The listing builds one solid part. Answer for the finished solid, in the listing's coordinates (mm). A direction names the side the tool comes from. Give positions to 0.01 mm unless a question says otherwise; leave off trailing zeros. Write each loop counter-clockwise with the first axis right and the second up, starting at its lowest first coordinate (ties: lowest second). Pieces come first, ordered by that corner, then holes.
```python
from build123d import *

# Parameters (mm, degrees)
SKETCH1_W           = 70
SKETCH1_H           = 30
BOSS_EXTRUDE1_DEPTH = 6
SKETCH2_R           = 1.25
CUT_EXTRUDE1_DEPTH  = 5
CUT_EXTRUDE2_START  = -5
SKETCH3_R           = 1.25
CUT_EXTRUDE2_DEPTH  = 5


with BuildPart() as part:
    # Sketch1 → Boss-Extrude1 (new body)
    with BuildSketch(Plane(origin=(0, 0, 0), x_dir=(1, 0, 0), z_dir=(0, 1, 0))):
        Rectangle(SKETCH1_W, SKETCH1_H)
    extrude(amount=BOSS_EXTRUDE1_DEPTH)

    # Sketch2 → Cut-Extrude1 (cut)
    with BuildSketch(Plane(origin=(35, 0, 0), x_dir=(0, 0, -1), z_dir=(1, 0, 0))):
        with Locations((11.5, 3)):
            Circle(SKETCH2_R)
        with Locations((-11.5, 3)):
            Circle(SKETCH2_R)
    extrude(amount=-CUT_EXTRUDE1_DEPTH, mode=Mode.SUBTRACT)

    # Sketch3 → Cut-Extrude2 (cut)
    with BuildSketch(Plane.ZY.offset(35).offset(CUT_EXTRUDE2_START)):
        with Locations(Location((-11.5, 3, 0), (0, 0, 180))):
            Circle(SKETCH3_R)
        with Locations(Location((11.5, 3, 0), (0, 0, 180))):
            Circle(SKETCH3_R)
    extrude(amount=CUT_EXTRUDE2_DEPTH, mode=Mode.SUBTRACT)


solid = part.part
```
Item 1: A cutting plane is placed at A-A, the plane z = 11.5. Give the vertices of the cut face in (x, y), plus the area to 3 significant figures.
Conclusion:
outline: (-35, 0) - (35, 0) - (35, 1.75) - (30, 1.75) - (30, 4.25) - (35, 4.25) - (35, 6) - (-35, 6) - (-35, 4.25) - (-30, 4.25) - (-30, 1.75) - (-35, 1.75) - close
area: 395 mm2
Item 2: A cutting plane is placed at C-C, the plane z = -11.75. Give the vertices of the cut face in (x, y), plus the area to 3 significant figures.
Conclusion:
outline: (-35, 0) - (35, 0) - (35, 1.78) - (30, 1.78) - (30, 4.22) - (35, 4.22) - (35, 6) - (-35, 6) - (-35, 4.22) - (-30, 4.22) - (-30, 1.78) - (-35, 1.78) - close
area: 396 mm2
Item 3: Each of these flat-tipped pins is pushed along its axis until it touches: P1, Ø5, axis at x = -13, z = 5.5, coming from the -Y side; P2, Ø2, axis at y = 3, z = 11.5, coming from the +X side; P3, Ø1.2, axis at y = 2.5, z = -11.5, coming from the -X side. Where does it stop, or does it pass through?
Conclusion:
P1: stops at y = 0
P2: stops at x = 30
P3: stops at x = -30
Item 4: Determine the mould class of faces 4 (the face through (0, 0, 0)), 5 (the face through (0, 3, -15)), 6 (the face through (-30, 3, -11)) for opening direction Z: pulls with the +Z half, pulls with the -Z half, needs draft (parallel to the pull), parting line crosses it, or undercut.
Conclusion:
face 4: needs draft
face 5: pulls with the -Z half
face 6: undercut
Item 5: Consider probe 1 along Z at (x, y) = (-32.55, 3); probe 2 along Y at (x, z) = (-32.3, 11.5). Determine where each line is inside the solid, lowest interval first.
Conclusion:
probe 1: z = -15 to -12.75, -10.25 to 10.25, 12.75 to 15
probe 2: y = 0 to 1.75, 4.25 to 6
Item 6: Which of the six approach directions +Z, -Z, +X, -X, +Y, -Y give full straight-line access (tool end or side, diameter ignored) to faces 1 (the face through (-30, 3, 12)), 2 (the face through (0, 6, 0)), 3 (the face through (32.53, 3.05, 12.75))?
Conclusion:
face 1: -X
face 2: +Z, -Z, +X, -X, +Y
face 3: +X
Item 7: A cutting plane is placed at B-B, the plane y = 3. Give the vertices of the cut face in (x, z), plus the area to 3 significant figures.
Conclusion:
outline: (-35, -15) - (35, -15) - (35, -12.75) - (30, -12.75) - (30, -10.25) - (35, -10.25) - (35, 10.25) - (30, 10.25) - (30, 12.75) - (35, 12.75) - (35, 15) - (-35, 15) - (-35, 12.75) - (-30, 12.75) - (-30, 10.25) - (-35, 10.25) - (-35, -10.25) - (-30, -10.25) - (-30, -12.75) - (-35, -12.75) - close
area: 2,050 mm2
